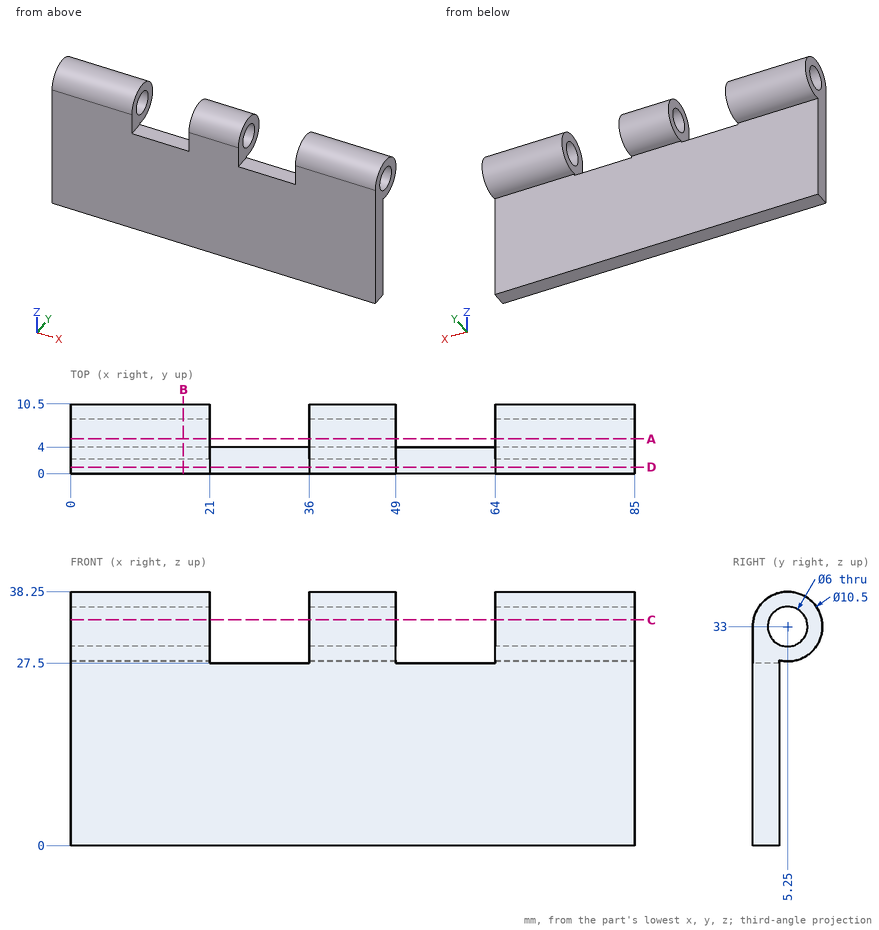
Design review of the part shown in the three views and the two pictorial views. Dimensions are in mm from the part's minimum x, y and z. Give positions to 0.01 mm unless a question says otherwise; leave off trailing zeros. Loops run counter-clockwise (first coordinate to the right, second up) from the corner with the lowest first, then second, coordinate; pieces in that order, holes last. Notation, with made-up numbers: (61, 14) -> (89, 14) arc R17 cw to (89, 22) -> close; hole circle Ø10 at (24.5, 27). An arc over 180 degrees is marked (long way). One line per item, written item: value.
Q1. We need section A-A on y = 5.25. Give the boundary of the cut face in (x, z).
Numbers:
outline: (0, 27.75) -> (21, 27.75) -> (21, 30) -> (0, 30) -> close; (0, 36) -> (21, 36) -> (21, 38.25) -> (0, 38.25) -> close; (36, 27.75) -> (49, 27.75) -> (49, 30) -> (36, 30) -> close; (36, 36) -> (49, 36) -> (49, 38.25) -> (36, 38.25) -> close; (64, 27.75) -> (85, 27.75) -> (85, 30) -> (64, 30) -> close; (64, 36) -> (85, 36) -> (85, 38.25) -> (64, 38.25) -> close
Q2. For L1, parallel to X at y = 2.5, z = 36.5; L2, parallel to Y at x = 80.25, z = 33; L3, parallel to Z at x = 20, y = 6.5, list the stretches that pass through material, from the lowest coordinate up.
Numbers:
L1: x = 0 to 21, 36 to 49, 64 to 85
L2: y = 0 to 2.25, 8.25 to 10.5
L3: z = 27.9 to 30.27, 35.73 to 38.1
Q3. We need section B-B on x = 17. Give the boundary of the cut face in (y, z).
Numbers:
outline: (0, 0) -> (4, 0) -> (4, 27.9) arc R5.25 ccw (long way) to (0, 33) -> close; hole circle Ø6 at (5.25, 33)
Q4. We need section C-C on z = 34. Give the boundary of the cut face in (x, y).
Numbers:
outline: (0, 0.1) -> (21, 0.1) -> (21, 2.42) -> (0, 2.42) -> close; (0, 8.08) -> (21, 8.08) -> (21, 10.4) -> (0, 10.4) -> close; (36, 0.1) -> (49, 0.1) -> (49, 2.42) -> (36, 2.42) -> close; (36, 8.08) -> (49, 8.08) -> (49, 10.4) -> (36, 10.4) -> close; (64, 0.1) -> (85, 0.1) -> (85, 2.42) -> (64, 2.42) -> close; (64, 8.08) -> (85, 8.08) -> (85, 10.4) -> (64, 10.4) -> close
Q5. We need section D-D on y = 1. Give the boundary of the cut face in (x, z).
Numbers:
outline: (0, 0) -> (85, 0) -> (85, 36.08) -> (64, 36.08) -> (64, 27.5) -> (49, 27.5) -> (49, 36.08) -> (36, 36.08) -> (36, 27.5) -> (21, 27.5) -> (21, 36.08) -> (0, 36.08) -> close
Q6. For pin 1 Ø2 at (x, y) = (66, 6) entering from -Z; pin 2 Ø5 at (y, z) = (5.25, 33) entering from +X; pin 3 Ø2 at (x, y) = (29.5, 1.5) entering from +Z; pin 4 Ø6 at (x, z) = (46, 13) entering from +Y, all flat-tipped, find the tip position at first contact; note any pin that passes through.
Numbers:
pin 1: stops at z = 27.75
pin 2: passes through
pin 3: stops at z = 27.5
pin 4: stops at y = 4
